Part model, mm, in its own coordinate system. A direction names the side the tool comes from. Round coordinates to 2 decimals unless told otherwise and drop trailing zeros. Loops run counter-clockwise (first coordinate to the right, second up) from the corner with the lowest first, then second, coordinate; pieces in that order, holes last. Notation, with made-up numbers: M 78,60.5 L 121,60.5 A25 ccw 121,99.5 Z; hole C -28,81 d1. An arc over 180 degrees is marked long. Put each result on its own line as item: value. Start each with the question number.
1) Slice it at A-A on y = 0. Give the cut face in (x, z), then the cut area to 3 significant figures.
2) Pull direction X, two halves, no side cores. Call faces 3 (the cylindrical face through (-1.08, -4.88, -1.74)), 4 (the cylindrical face through (-4.75, 0.04, -0.01)), 5 (the flat face through (2, -2, -2.5)): +X half, -X half, draft (parallel to the pull), parting line (faces both ways), or undercut.
3) Probe line 1 along Z through (x, y) = (3.75, -1.75); line 2 along Y through (x, z) = (0, -1.5); line 3 along Y through (x, z) = (3, -0.8). List the from-to ranges inside material, lowest first.
4) Drop flat-ended pins along their axis: pin 1 Ø2 at (y, z) = (1.5, 1.5) entering from -X; pin 2 Ø2 at (y, z) = (2, 0.5) entering from +X. Give the stop position or say it passes through.
5) Slice it at C-C on z = -0.8. Give the cut face in (x, y).
6) Which spindle directions (+Z, -Z, +X, -X, +Y, -Y) get a long thin tool onto all of the face, cutting with end or side? Do faces 1 (the cylindrical face through (-0.13, -2.76, -0.01)), 2 (the cylindrical face through (-0.54, -2.44, 1.74)). Say none if no direction does.
7) Slice it at D-D on y = -1.5. Give the cut face in (x, z).
```python
from build123d import *

# Parameters (mm, degrees)
BOSS_EXTRUDE1_START = 1
SKETCH4_4_R         = 5
SKETCH4_4_R_2       = 2.5
BOSS_EXTRUDE1_DEPTH = 1.5
BOSS_EXTRUDE2_START = -1
SKETCH_4_4_R        = 5
SKETCH_4_4_R_2      = 2.5
BOSS_EXTRUDE2_DEPTH = 1.5
SKETCH8_R           = 1
BOSS_EXTRUDE3_DEPTH = 2


with BuildPart() as part:
    # Sketch4<4> → Boss-Extrude1 (new body)
    with BuildSketch(Plane.XY.offset(BOSS_EXTRUDE1_START)):
        Circle(SKETCH4_4_R)
        Circle(SKETCH4_4_R_2, mode=Mode.SUBTRACT)
    extrude(amount=BOSS_EXTRUDE1_DEPTH)



with BuildPart() as body_2:
    # 草图4<4> → Boss-Extrude2 (new body)
    with BuildSketch(Plane.XY.offset(BOSS_EXTRUDE2_START)):
        Circle(SKETCH_4_4_R)
        Circle(SKETCH_4_4_R_2, mode=Mode.SUBTRACT)
    extrude(amount=-BOSS_EXTRUDE2_DEPTH)


with BuildPart() as part_1:
    add(part.part)

    add(body_2.part)  # Boss-Extrude3 merges body 2
    # Sketch8 → Boss-Extrude3 (add)
    with BuildSketch(Plane.XY.offset(-1)):
        with Locations((0, 3.75)):
            Circle(SKETCH8_R)
        with Locations((2.651650429, 2.651650429)):
            Circle(SKETCH8_R)
        with Locations((3.75, 0)):
            Circle(SKETCH8_R)
        with Locations((2.651650429, -2.651650429)):
            Circle(SKETCH8_R)
        with Locations((0, -3.75)):
            Circle(SKETCH8_R)
        with Locations((-2.651650429, -2.651650429)):
            Circle(SKETCH8_R)
        with Locations((-3.75, 0)):
            Circle(SKETCH8_R)
        with Locations((-2.651650429, 2.651650429)):
            Circle(SKETCH8_R)
    extrude(amount=BOSS_EXTRUDE3_DEPTH)


solid = part_1.part
```
Recorded:
1. outline: M -5,-2.5 L -2.5,-2.5 L -2.5,-1 L -2.75,-1 L -2.75,1 L -2.5,1 L -2.5,2.5 L -5,2.5 L -5,1 L -4.75,1 L -4.75,-1 L -5,-1 Z; M 2.5,-2.5 L 5,-2.5 L 5,-1 L 4.75,-1 L 4.75,1 L 5,1 L 5,2.5 L 2.5,2.5 L 2.5,1 L 2.75,1 L 2.75,-1 L 2.5,-1 Z
1. area: 23.0 mm2
2. face 3: parting line
2. face 4: undercut
2. face 5: draft
3. line 1: z = -2.5 to -1, 1 to 2.5
3. line 2: y = -5 to -2.5, 2.5 to 5
3. line 3: y = -3.59 to -1.71, -0.66 to 0.66, 1.71 to 3.59
4. pin 1: stops at x = -4.97
4. pin 2: stops at x = 4.87
5. outline: C -3.75,0 d2; C -2.65,-2.65 d2; C -2.65,2.65 d2; C 0,-3.75 d2; C 0,3.75 d2; C 2.65,-2.65 d2; C 2.65,2.65 d2; C 3.75,0 d2
6. face 1: none
6. face 2: +Z, -Z
7. outline: M -4.77,-2.5 L -2,-2.5 L -2,-1 L -4.77,-1 Z; M -4.77,1 L -2,1 L -2,2.5 L -4.77,2.5 Z; M 2,-2.5 L 4.77,-2.5 L 4.77,-1 L 2,-1 Z; M 2,1 L 4.77,1 L 4.77,2.5 L 2,2.5 Z
